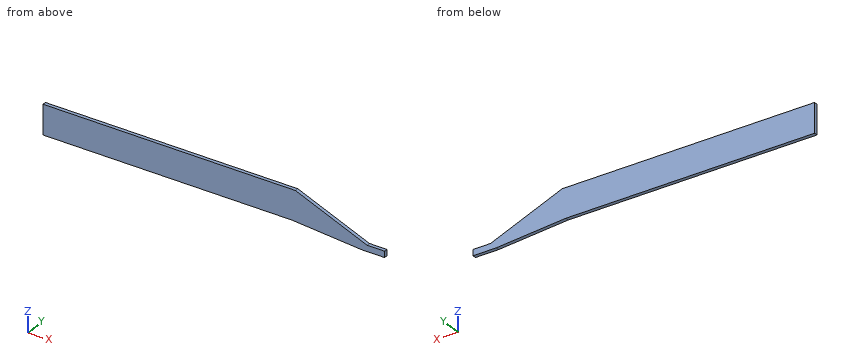
from build123d import *

# Parameters (mm, degrees)
BOSS_EXTRUDE1_DEPTH = 0.2


with BuildPart() as part:
    # Sketch1 → Boss-Extrude1 (new body)
    with BuildSketch(Plane(origin=(0, 0, 0), x_dir=(1, 0, 0), z_dir=(0, 1, 0))):
        Polygon((19.5, 1.67), (18.5, 1.67), (14.40778992, 0), (0, 0), (0, 1.7), (14.2, 1.7), (18.177225926, 2.02), (19.5, 2.02), align=None)
    extrude(amount=BOSS_EXTRUDE1_DEPTH)


solid = part.part
Could you check a few things on this model? Use its own coordinates, in mm. Coordinates: 2 decimals unless noted, no trailing zeros. Order: outer loops, then holes, each group sorted by start corner. A loop starts at its lowest first (then second) coordinate and runs counter-clockwise, first axis right, second up. Notation, with made-up numbers: (12, 70.25) - (24, 70.25) arc R19 cw to (24, 96.25) - close; hole circle Ø1 at (19.25, 18). An arc over 180 degrees is marked (long way). Answer in a Markdown table with one row per item. Add a question column.
(1) I need wall thicknesses on L1, parallel to Z at x = 2, y = 0.15; L2, parallel to X at y = 0.15, z = -0.65; L3, parallel to X at y = 0.1, z = -1.4. Which ranges of each line are inside material? Lowest first, please.
(2) If we section it at C-C, the plane z = -0.4: Please give me the cut outline in (x, y).
(3) If we section it at B-B, the plane x = 10: Please give me the cut outline in (y, z), then the cut area to 3 significant figures.
(4) If we section it at A-A, the plane y = 0.15: Please give me the cut outline in (x, z).
Results are:
| question | item | result |
|---|---|---|
| 1 | L1 | z = -1.7 to 0 |
| 1 | L2 | x = 0 to 16 |
| 1 | L3 | x = 0 to 17.84 |
| 2 | outline | (0, 0) - (15.39, 0) - (15.39, 0.2) - (0, 0.2) - close |
| 3 | outline | (0, -1.7) - (0.2, -1.7) - (0.2, 0) - (0, 0) - close |
| 3 | area | 0.340 mm2 |
| 4 | outline | (0, -1.7) - (14.2, -1.7) - (18.18, -2.02) - (19.5, -2.02) - (19.5, -1.67) - (18.5, -1.67) - (14.41, 0) - (0, 0) - close |
